from build123d import *

# Parameters (mm, degrees)
EXTRUDE_1_DEPTH = 2
EXTRUDE_2_DEPTH = 4


with BuildPart() as part:
    # 草图1 → 凸台-拉伸1 (new body)
    with BuildSketch(Plane.XY):
        with BuildLine():
            Line((137.488957816, 148.560574876), (148.33581351, 109.973924886))
            ThreePointArc((148.33581351, 109.973924886), (149.830188599, 108.129149559), (152.197376559, 107.948113442))
            Line((152.197376559, 107.948113442), (153.12452466, 108.266185323))
            ThreePointArc((153.12452466, 108.266185323), (154.455434588, 109.182984766), (155.117593814, 110.657226135))
            ThreePointArc((155.117593814, 110.657226135), (175.157111586, 151.143900213), (214.998888251, 172.436760111))
            ThreePointArc((214.998888251, 172.436760111), (217.048600661, 173.871762608), (217.297595906, 176.361452247))
            Line((217.297595906, 176.361452247), (216.233642795, 179.462770427))
            ThreePointArc((216.233642795, 179.462770427), (214.647795853, 181.215617846), (212.284799547, 181.275892717))
            Line((212.284799547, 181.275892717), (139.265834382, 152.159042969))
            ThreePointArc((139.265834382, 152.159042969), (137.68708728, 150.700674405), (137.488957816, 148.560574876))
        make_face()
    extrude(amount=-EXTRUDE_1_DEPTH)

    # 草图2 → 凸台-拉伸2 (add)
    with BuildSketch(Plane.XY):
        with BuildLine():
            Line((153.773524821, 106.374413986), (152.84637672, 106.056342105))
            ThreePointArc((152.84637672, 106.056342105), (148.901063453, 106.358068967), (146.410438304, 109.432694512))
            Line((146.410438304, 109.432694512), (135.563582611, 148.019344502))
            ThreePointArc((135.563582611, 148.019344502), (135.893798384, 151.586177051), (138.525043553, 154.016791324))
            Line((138.525043553, 154.016791324), (211.544008718, 183.133641072))
            ThreePointArc((211.544008718, 183.133641072), (215.482335894, 183.033182953), (218.125414132, 180.111770588))
            Line((218.125414132, 180.111770588), (219.189367243, 177.010452408))
            ThreePointArc((219.189367243, 177.010452408), (218.774375168, 172.860969677), (215.358187818, 170.469298848))
            ThreePointArc((215.358187818, 170.469298848), (176.593215928, 149.75192165), (157.095306744, 110.359482007))
            ThreePointArc((157.095306744, 110.359482007), (155.991708034, 107.902413058), (153.773524821, 106.374413986))
        make_face()
    extrude(amount=EXTRUDE_2_DEPTH)


solid = part.part
Read the model definition and answer for the solid it produces. Units are mm, in the model's axes. A direction names the side the tool comes from. Coordinates: 2 decimals unless noted, no trailing zeros. Order: outer loops, then holes, each group sorted by start corner. A loop starts at its lowest first (then second) coordinate and runs counter-clockwise, first axis right, second up. Notation, with made-up numbers: M 65,15.25 L 76,15.25 A26 cw 76,46.25 Z; hole C 56,36 d9. An arc over 180 degrees is marked long. Put each result on its own line as item: value. Start each with the question number.
Item 1: Given pin 1 Ø2 at (x, z) = (189.5, 1.5) entering from +Y; pin 2 Ø1 at (x, z) = (185, 1) entering from +Y; pin 3 Ø2 at (y, z) = (115, 1.5) entering from +X, each flat-ended and moving along its own axis, determine where each tip first touches the part or whether it passes through.
Item 2: Consider probe 1 along Z at (x, y) = (190, 161); probe 2 along Y at (x, z) = (162.5, 1.45); probe 3 along Y at (x, z) = (168, 2.75). Determine where each line is inside the solid, lowest interval first. Write a range as [from, to].
Item 3: Section A-A, the plane z = 2.15 is taken. Determine the outline of the cut face in (x, y), plus the area to 3 significant figures.
Item 4: Section C-C, the plane x = 162.5 is taken. Determine the outline of the cut face in (y, z), plus the area to 3 significant figures.
Item 5: Section B-B, the plane y = 149.5 is taken. Determine the outline of the cut face in (x, z), plus the area to 3 significant figures.
Item 6: For faces 1 (the face through (178, 153, 0)), 2 (the face through (217.03, 173.84, -0.99)), 3 (the face through (149.8, 108.145, -0.986)), 4 (the face through (137.7, 150.73, -0.99)), determine the directions among +Z, -Z, +X, -X, +Y, -Y from which every point of the face is accessible in a straight line to the end or side of a thin tool.
Computed:
1. pin 1: stops at y = 174.74
1. pin 2: stops at y = 172.75
1. pin 3: stops at x = 158.18
2. probe 1: z = [0, 4]
2. probe 2: y = [128.89, 163.58]
2. probe 3: y = [138.99, 165.77]
3. outline: M 135.56,148.02 L 146.41,109.43 A5 ccw 152.85,106.06 L 153.77,106.37 A5 ccw 157.1,110.36 A72 cw 215.36,170.47 A5 ccw 219.19,177.01 L 218.13,180.11 A5 ccw 211.54,183.13 L 138.53,154.02 A5 ccw Z
3. area: 2,020 mm2
4. outline: M 128.89,0 L 133.51,0 L 133.51,-2 L 161.42,-2 L 161.42,0 L 163.58,0 L 163.58,4 L 128.89,4 Z
4. area: 195 mm2
5. outline: M 135.38,0 L 137.38,0 L 137.38,-2 L 173.61,-2 L 173.61,0 L 176.35,0 L 176.35,4 L 135.38,4 Z
5. area: 236 mm2
6. face 1: -Z
6. face 2: -Z, +X
6. face 3: -Z, -Y
6. face 4: -Z, -X
